Check sheet for the modelled part. Datum: model origin and axes. Units: mm. A direction names the side the tool comes from. Coordinates: 2 decimals unless noted, no trailing zeros. Loops run counter-clockwise (first coordinate to the right, second up) from the corner with the lowest first, then second, coordinate; pieces in that order, holes last. Notation, with made-up numbers: M 61.25,43 L 84.25,43 A24 ccw 84.25,65 Z; hole C -10.5,8 d4. An arc over 180 degrees is marked long. Use CSV: the item, a comma, the result in double quotes. Start each with the question number.
(1) Section check C-C on x = 12. Record the cut outline in (y, z).
(2) Set-up check for faces 1 (the flat face through (-1, 15, -87.5)), 2 (the flat face through (-1, 10, -4)): record each of +Z, -Z, +X, -X, +Y, -Y from which the full face is reachable in a straight line by a thin tool's end or side.
(3) Draft check along X on faces 3 (the cylindrical face through (-40.31, 4.93, 0.96)), 4 (the flat face through (-55, 8, -28)), 5 (the flat face through (1, 20, -77.5)), 6 (the flat face through (55, 8, -28)). Enter one of: pulls with the +X half, pulls with the -X half, needs draft (parallel to the pull), parting line crosses it, or undercut.
(4) Section check A-A on x = -38. Record the cut outline in (y, z), and give its area (3 significant figures).
(5) Section check D-D on y = 13. Record the cut outline in (x, z), and give its area (3 significant figures).
(6) Section check B-B on z = -27. Record the cut outline in (x, y), and give its area (3 significant figures).
(7) Go/stop test with flat-tipped pins: pin 1 Ø1.5 at (x, y) = (-19, 11) entering from +Z; pin 2 Ø4.5 at (x, z) = (-38, -27) entering from -Y; pin 3 Ø1 at (x, z) = (33, -40) entering from +Y. Record where each tip stops, or that it passes through.
(8) Scan lines: line 1 (X direction, y = 4.5, z = -27); line 2 (Z direction, x = 38, y = 4.5); line 3 (Z direction, x = -8.5, y = 21). Record each from-to range of solid material in increasing order.
from build123d import *

# Parameters (mm, degrees)
SKETCH_2_W         = 110
SKETCH_2_H         = 135
EXTRUDE_1_DEPTH    = 10
HOLE_WIZARD_M6_1_D = 5
SKETCH_11_W        = 110
SKETCH_11_H        = 20
EXTRUDE_6_DEPTH    = 10
SKETCH_15_W        = 110
SKETCH_15_H        = 30
EXTRUDE_7_DEPTH    = 10


with BuildPart() as part:
    # 草图2 → 凸台-拉伸1 (new body)
    with BuildSketch(Plane(origin=(0, 0, 0), x_dir=(1, 0, 0), z_dir=(0, 1, 0))):
        Rectangle(SKETCH_2_W, SKETCH_2_H)
    extrude(amount=EXTRUDE_1_DEPTH)

    # M6 螺纹孔1 (through all)
    with Locations(Plane(origin=(0, 10, 0), x_dir=(1, 0, 0), z_dir=(0, 1, 0))):
        with Locations((-38, 27), (-38, 0), (38, 0), (-38, -27), (38, -27), (38, 27)):
            Hole(HOLE_WIZARD_M6_1_D / 2)

    # 草图11 → 凸台-拉伸6 (add)
    with BuildSketch(Plane.XZ):
        with Locations((0, -77.5)):
            Rectangle(SKETCH_11_W, SKETCH_11_H)
    extrude(amount=-EXTRUDE_6_DEPTH)

    # 草图15 → 凸台-拉伸7 (add)
    with BuildSketch(Plane(origin=(0, 0, -87.5), x_dir=(-1, 0, 0), z_dir=(0, 0, -1))):
        with Locations((0, 15)):
            Rectangle(SKETCH_15_W, SKETCH_15_H)
    extrude(amount=-EXTRUDE_7_DEPTH)


solid = part.part
Outcome:
1,outline,"M 0,-87.5 L 30,-87.5 L 30,-77.5 L 10,-77.5 L 10,67.5 L 0,67.5 Z"
2,face 1,"-Z, +X, -X, +Y, -Y"
2,face 2,"+Z, +X, -X, +Y"
3,face 3,"undercut"
3,face 4,"pulls with the -X half"
3,face 5,"needs draft"
3,face 6,"pulls with the +X half"
4,outline,"M 0,-87.5 L 30,-87.5 L 30,-77.5 L 10,-77.5 L 10,-29.5 L 0,-29.5 Z; M 0,-24.5 L 10,-24.5 L 10,-2.5 L 0,-2.5 Z; M 0,2.5 L 10,2.5 L 10,24.5 L 0,24.5 Z; M 0,29.5 L 10,29.5 L 10,67.5 L 0,67.5 Z"
4,area,"1,600 mm²"
5,outline,"M -55,-87.5 L 55,-87.5 L 55,-77.5 L -55,-77.5 Z"
5,area,"1,100 mm²"
6,outline,"M -55,0 L -40.5,0 L -40.5,10 L -55,10 Z; M -35.5,0 L 35.5,0 L 35.5,10 L -35.5,10 Z; M 40.5,0 L 55,0 L 55,10 L 40.5,10 Z"
6,area,"1,000 mm²"
7,pin 1,"stops at z = -77.5"
7,pin 2,"passes through"
7,pin 3,"stops at y = 10"
8,line 1,"x = -55 to -40.5, -35.5 to 35.5, 40.5 to 55"
8,line 2,"z = -87.5 to -29.5, -24.5 to -2.5, 2.5 to 24.5, 29.5 to 67.5"
8,line 3,"z = -87.5 to -77.5"
